Build history of the part. All positions in model axes, mm. A direction names the side the tool comes from. Give positions to 0.01 mm unless a question says otherwise; leave off trailing zeros. Write each loop counter-clockwise with the first axis right and the second up, starting at its lowest first coordinate (ties: lowest second). Pieces come first, ordered by that corner, then holes. Notation, with made-up numbers: (60, 58) -> (109, 58) arc R25 ccw to (109, 78) -> close; hole circle Ø1 at (-26.75, 38). An arc over 180 degrees is marked (long way). One line per question, with ' | ' between items. Start each with the question number.
(1) Pull direction X, two halves, no side cores. Call faces 1 (the flat face through (21, 53, 7.5)), 2 (the cylindrical face through (-0.508, 129.094, 0.105)), 3 (the flat face through (19.1, 54, 0)): released by +X, released by -X, zero draft, split by the parting line, or undercut.
(2) Tool access for faces 4 (the cylindrical face through (-0.42, 125.095, 0.105)), 5 (the cylindrical face through (0.508, -23.094, 0.105)): list every direction of +Z, -Z, +X, -X, +Y, -Y with a clear straight run to the whole face (end or side of a thin tool).
(3) Band-saw the part on A-A, the plane z = 0.25. Give the cut face in (x, y).
(4) Drill centre lines: probe 1 along X at (y, z) = (99, -6.5); probe 2 along X at (y, z) = (-7, -2.25); probe 3 along Y at (x, z) = (-5.5, -7). Where is each one in solid material? Low to high. Write a range as from..to.
(5) Pin check, flat tip, straight feed: P1, Ø3, axis at y = 106.5, z = -4.5, coming from the -X side. Stop position of the tip, or through.
(6) Band-saw the part on C-C, the plane x = 0. Give the cut face in (y, z).
(7) Band-saw the part on B-B, the plane y = 16. Give the cut face in (x, z).
from build123d import *

# Parameters (mm, degrees)
EXTRUDE_1_DEPTH = 7.5


with BuildPart() as part:
    # 草图2 → 拉伸-薄壁1 (new, symmetric)
    with BuildSketch(Plane.XY):
        with BuildLine():
            Line((23.1, 106), (23.1, 0))
            ThreePointArc((23.1, 0), (0, -23.1), (-23.1, 0))
            Line((-23.1, 0), (-23.1, 106))
            ThreePointArc((-23.1, 106), (0, 129.1), (23.1, 106))
        make_face()
        with BuildLine():
            Line((19.1, 106), (19.1, 0))
            ThreePointArc((19.1, 0), (0, -19.1), (-19.1, 0))
            Line((-19.1, 0), (-19.1, 106))
            ThreePointArc((-19.1, 106), (0, 125.1), (19.1, 106))
        make_face(mode=Mode.SUBTRACT)
    extrude(amount=EXTRUDE_1_DEPTH, both=True)


solid = part.part
Results:
1) face 1: zero draft | face 2: split by the parting line | face 3: undercut
2) face 4: +Z, -Z | face 5: +Z, -Z, -Y
3) outline: (-23.1, 0) arc R23.1 ccw to (23.1, 0) -> (23.1, 106) arc R23.1 ccw to (-23.1, 106) -> close; hole (-19.1, 0) arc R19.1 ccw to (19.1, 0) -> (19.1, 106) arc R19.1 ccw to (-19.1, 106) -> close
4) probe 1: x = -23.1..-19.1, 19.1..23.1 | probe 2: x = -22.01..-17.77, 17.77..22.01 | probe 3: y = -22.44..-18.29, 124.29..128.44
5) P1: stops at x = -23.1
6) outline: (-23.1, -7.5) -> (-19.1, -7.5) -> (-19.1, 7.5) -> (-23.1, 7.5) -> close; (125.1, -7.5) -> (129.1, -7.5) -> (129.1, 7.5) -> (125.1, 7.5) -> close
7) outline: (-23.1, -7.5) -> (-19.1, -7.5) -> (-19.1, 7.5) -> (-23.1, 7.5) -> close; (19.1, -7.5) -> (23.1, -7.5) -> (23.1, 7.5) -> (19.1, 7.5) -> close
